```python
from build123d import *
from OCP.BRepFilletAPI import BRepFilletAPI_MakeChamfer

# Parameters (mm, degrees)
SKETCH1_W             = 45
SKETCH1_H             = 50
BOSS_EXTRUDE1_DEPTH   = 2
SKETCH2_W             = 3.2
SKETCH2_H             = 3.8
CUT_EXTRUDE1_DEPTH    = 34.693471178
SKETCH3_W             = 2
SKETCH3_H             = 18
CUT_EXTRUDE2_DEPTH    = 34.693471178
SKETCH4_W             = 2
SKETCH4_H             = 4
CUT_EXTRUDE3_DEPTH    = 1
CUT_EXTRUDE4_DEPTH    = 3
SKETCH6_W             = 46.8
SKETCH6_H             = 10
CUT_EXTRUDE5_DEPTH    = 1
CHAMFER1_SIZE         = 15
CHAMFER1_SIZE2        = 5
CHAMFER2_SIZE         = 5
CHAMFER2_SIZE2        = 15
SKETCH8_W             = 45
SKETCH8_H             = 2
BOSS_EXTRUDE2_DEPTH   = 3
SKETCH7_R             = 1.75
CUT_EXTRUDE6_DEPTH    = 36.975686234
FILLET2_R             = 15
CHAMFER4_SIZE         = 2
CHAMFER4_SIZE2        = 0.2
SKETCH10_W            = 4.825824379
SKETCH10_H            = 2.951447422
CUT_EXTRUDE7_DEPTH    = 36.975686234
CHAMFER5_SIZE         = 1
M2_TAPPED_HOLE1_D     = 1.6
M2_TAPPED_HOLE1_DEPTH = 5.2
M2_TAPPED_HOLE1_TIP   = 0.480688495


with BuildPart() as part:
    # Sketch1 → Boss-Extrude1 (new body)
    with BuildSketch(Plane(origin=(0, 0, 0), x_dir=(1, 0, 0), z_dir=(0, 1, 0))):
        Rectangle(SKETCH1_W, SKETCH1_H)
    extrude(amount=BOSS_EXTRUDE1_DEPTH)

    # Sketch2 → Cut-Extrude1 (cut, through all)
    with BuildSketch(Plane(origin=(0, 2, 0), x_dir=(1, 0, 0), z_dir=(0, 1, 0))):
        with Locations((0.7, 9.95)):
            Rectangle(SKETCH2_W, SKETCH2_H)
    extrude(amount=-CUT_EXTRUDE1_DEPTH, mode=Mode.SUBTRACT)

    # Sketch3 → Cut-Extrude2 (cut, through all)
    with BuildSketch(Plane(origin=(0, 2, 0), x_dir=(1, 0, 0), z_dir=(0, 1, 0))):
        with Locations((-2.75, 12)):
            Rectangle(SKETCH3_W, SKETCH3_H)
    extrude(amount=-CUT_EXTRUDE2_DEPTH, mode=Mode.SUBTRACT)

    # Sketch4 → Cut-Extrude3 (cut)
    with BuildSketch(Plane.XZ):
        with Locations((-2.75, -23)):
            Rectangle(SKETCH4_W, SKETCH4_H)
    extrude(amount=-CUT_EXTRUDE3_DEPTH, mode=Mode.SUBTRACT)

    # Sketch5 → Cut-Extrude4 (cut)
    with BuildSketch(Plane(origin=(0, 2, 0), x_dir=(1, 0, 0), z_dir=(0, 1, 0))):
        with BuildLine():
            Line((-0.9, 8.05), (26.461433113, 8.05))
            Line((26.461433113, 8.05), (36.248351242, 8.05))
            ThreePointArc((36.248351242, 8.05), (17.674175621, -14.95), (-0.9, 8.05))
        make_face()
    extrude(amount=-CUT_EXTRUDE4_DEPTH, mode=Mode.SUBTRACT)

    # Sketch6 → Cut-Extrude5 (cut)
    with BuildSketch(Plane(origin=(0, 2, 0), x_dir=(1, 0, 0), z_dir=(0, 1, 0))):
        with Locations((-0.9, 9.95)):
            Rectangle(SKETCH6_W, SKETCH6_H)
    extrude(amount=-CUT_EXTRUDE5_DEPTH, mode=Mode.SUBTRACT)

    # Chamfer1: one chamfer whose edges measure the first distance from different faces: ONE call of the kernel's chamfer builder (chamfer() names one face for all edges)
    chamfer1_edges_1 = [part.edges().sort_by_distance(p)[0] for p in [
        (-22.5, 1.5, -14.95),
    ]]
    chamfer1_side_1 = [part.faces().sort_by_distance(p)[0] for p in [
        (-13.125, 1.5, -14.95),
    ]]
    chamfer1_edges_2 = [part.edges().sort_by_distance(p)[0] for p in [
        (-22.5, 1.5, -4.95),
    ]]
    chamfer1_side_2 = [part.faces().sort_by_distance(p)[0] for p in [
        (-13.125, 1.5, -4.95),
    ]]
    chamfer1 = BRepFilletAPI_MakeChamfer(part.part.solid().wrapped)
    for e in chamfer1_edges_1:
        chamfer1.Add(CHAMFER1_SIZE, CHAMFER1_SIZE2, e.wrapped, chamfer1_side_1[0].wrapped)  # the first distance lies on this face
    for e in chamfer1_edges_2:
        chamfer1.Add(CHAMFER1_SIZE, CHAMFER1_SIZE2, e.wrapped, chamfer1_side_2[0].wrapped)  # the first distance lies on this face
    add(Compound.cast(chamfer1.Shape()), mode=Mode.REPLACE)

    # Chamfer2
    chamfer2_edges = [part.edges().sort_by_distance(p)[0] for p in [
        (22.5, 1.5, -14.95),
    ]]
    chamfer2_side = [part.faces().sort_by_distance(p)[0] for p in [
        (22.5, 0.872222222, -17.809166667),
    ]]
    chamfer(chamfer2_edges, length=CHAMFER2_SIZE, length2=CHAMFER2_SIZE2, reference=chamfer2_side[0])

    # Sketch8 → Boss-Extrude2 (add)
    with BuildSketch(Plane.XY.offset(25)):
        with Locations((0, 1)):
            Rectangle(SKETCH8_W, SKETCH8_H)
    extrude(amount=BOSS_EXTRUDE2_DEPTH)

    # Sketch7 → Cut-Extrude6 (cut, through all)
    with BuildSketch(Plane(origin=(0, 2, 0), x_dir=(1, 0, 0), z_dir=(0, 1, 0))):
        with Locations(Location((-17.5, 21, 0), (0, 0, 270))):
            Circle(SKETCH7_R)
        with Locations(Location((17.5, 21, 0), (0, 0, 90))):
            Circle(SKETCH7_R)
        with Locations(Location((17.5, -24, 0), (0, 0, 270))):
            Circle(SKETCH7_R)
        with Locations(Location((-17.5, -24, 0), (0, 0, 90))):
            Circle(SKETCH7_R)
    extrude(amount=-CUT_EXTRUDE6_DEPTH, mode=Mode.SUBTRACT)

    # Fillet2
    fillet2_edges = [part.edges().sort_by_distance(p)[0] for p in [
        (22.5, 0.5, -8.05),
    ]]
    fillet(fillet2_edges, radius=FILLET2_R)

    # Chamfer4
    chamfer4_edges = [part.edges().sort_by_distance(p)[0] for p in [
        (10.375, 0, -25),
        (-13.125, 0, -25),
    ]]
    chamfer4_side = [part.faces().sort_by_distance(p)[0] for p in [
        (-3.590988943, 0, 2.118757262),
    ]]
    chamfer(chamfer4_edges, length=CHAMFER4_SIZE, length2=CHAMFER4_SIZE2, reference=chamfer4_side[0])

    # Sketch10 → Cut-Extrude7 (cut, through all)
    with BuildSketch(Plane(origin=(0, 2, 0), x_dir=(1, 0, 0), z_dir=(0, 1, 0))):
        with Locations((20.087087811, -13.474276289)):
            Rectangle(SKETCH10_W, SKETCH10_H)
    extrude(amount=-CUT_EXTRUDE7_DEPTH, mode=Mode.SUBTRACT)

    # Chamfer5
    chamfer5_edges = [part.edges().sort_by_distance(p)[0] for p in [
        (22.5, 1.1, -25),
    ]]
    chamfer(chamfer5_edges, length=CHAMFER5_SIZE)

    # M2 Tapped Hole1
    with Locations(Plane(origin=(0, 2, 0), x_dir=(1, 0, 0), z_dir=(0, 1, 0))):
        with Locations((-6.9, -7.5), (-6.9, -2.5)):
            Hole(M2_TAPPED_HOLE1_D / 2, depth=M2_TAPPED_HOLE1_DEPTH)
            with Locations((0, 0, -(M2_TAPPED_HOLE1_DEPTH + M2_TAPPED_HOLE1_TIP / 2))):  # 118° drill point
                Cone(0, M2_TAPPED_HOLE1_D / 2, M2_TAPPED_HOLE1_TIP, mode=Mode.SUBTRACT)


solid = part.part
```
For this review, take the finished solid that the model builds, in its own axes (mm). A direction names the side the tool comes from. Round coordinates to 2 decimals unless told otherwise and drop trailing zeros. Loops run counter-clockwise (first coordinate to the right, second up) from the corner with the lowest first, then second, coordinate; pieces in that order, holes last.
(1) Tool access review of faces 5 (the cylindrical face through (19.88, 0.57, -14.58)), 6 (the flat face through (-3, 1, -23)), 7 (the flat face through (14.723, 1.507, -17.358)), 8 (the flat face through (-3, 1, -3)): name each direction out of +Z, -Z, +X, -X, +Y, -Y from which nothing blocks a thin tool from reaching the whole face with its end or side.
Returned:
face 5: +X, +Y, -Y
face 6: -Z, -Y
face 7: +X, +Y
face 8: +Y, -Y
(2) Mouldability with a two-part tool opening along X and no side actions: class faces 1 (the flat face through (-15.105, 1.493, -17.485)), 2 (the cylindrical face through (3.04, 1.01, 8.07)), 3 (the flat face through (0, 1, 28)), 4 (the cylindrical face through (16.32, 1.01, -19.71)) as released by +X, released by -X, zero draft, split by the parting line, or undercut.
Returned:
face 1: released by -X
face 2: released by +X
face 3: zero draft
face 4: undercut
(3) Clearance check with flat-ended pins moving along their axes: P1, Ø0.5, axis at y = 0.5, z = -10, coming from the +X side; P2, Ø3, axis at x = 3, z = -9, coming from the +Y side; P3, Ø1, axis at y = 0.5, z = -19.5, coming from the +X side; P4, Ø12, axis at x = 6, z = -10, coming from the +Y side. State where each tip first meets the part, or that it passes through.
Returned:
P1: stops at x = 15.32
P2: stops at y = 1
P3: stops at x = 22.19
P4: stops at y = 2
(4) We need section C-C (x = -6.9). Give the boundary of the cut face in (y, z), plus the area to 3 significant figures.
Returned:
outline: (0, -23) - (0.2, -25) - (2, -25) - (2, -14.95) - (1, -14.95) - (1, -4.95) - (2, -4.95) - (2, 1.7) - (0, 1.7) - close; (0, 3.3) - (2, 3.3) - (2, 6.7) - (0, 6.7) - close; (0, 8.3) - (2, 8.3) - (2, 28) - (0, 28) - close
area: 89.4 mm2
(5) We need section A-A (y = 1.55). State how many separate pieces and enclosed holes the cut face has, plus the area to 3 significant figures.
Returned:
separate pieces: 2
enclosed holes: 6
area: 1,370 mm2
(6) We need section D-D (z = 2.5). Give the boundary of the cut face in (x, y).
Returned:
outline: (-22.5, 0) - (-7.7, 0) - (-7.7, 2) - (-22.5, 2) - close; (-6.1, 0) - (-0.16, 0) - (-0.16, 2) - (-6.1, 2) - close
(7) Wall thickness on line 1 along X through (y, z) = (1.25, 24); line 2 along Z through (x, y) = (-7, 1.35); line 3 along Z through (x, y) = (-4, 1.7): over which ranges is each line inside the solid? List them lowest first.
Returned:
line 1: x = -22.5 to -19.25, -15.75 to 15.75, 19.25 to 22.5
line 2: z = -25 to -14.95, -4.95 to 1.71, 3.29 to 6.71, 8.29 to 28
line 3: z = -25 to -14.95, -4.95 to 28
(8) We need section B-B (z = 24). Give the boundary of the cut face in (x, y).
Returned:
outline: (-22.5, 0) - (-19.25, 0) - (-19.25, 2) - (-22.5, 2) - close; (-15.75, 0) - (15.75, 0) - (15.75, 2) - (-15.75, 2) - close; (19.25, 0) - (22.5, 0) - (22.5, 2) - (19.25, 2) - close
